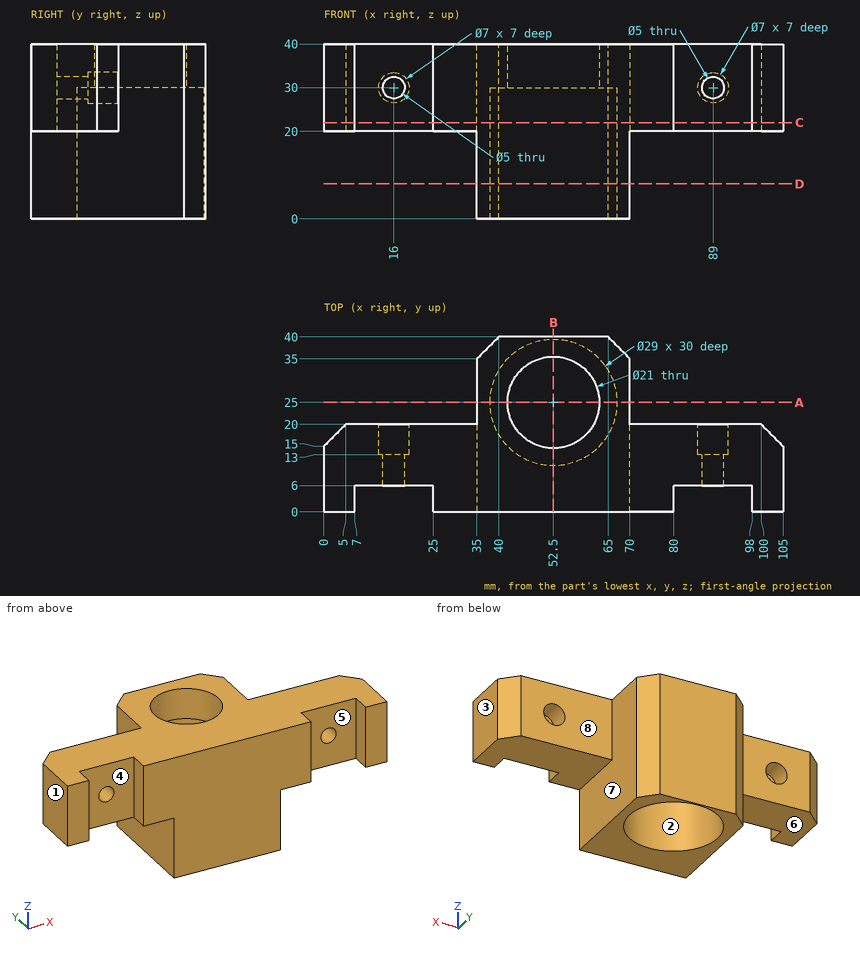
Check sheet for the drawn part. Datum: minimum x, y, z corner. Units: mm. A direction names the side the tool comes from. Round coordinates to 2 decimals unless told otherwise and drop trailing zeros. Order: outer loops, then holes, each group sorted by start corner. A loop starts at its lowest first (then second) coordinate and runs counter-clockwise, first axis right, second up.
1. Access from +Z, -Z, +X, -X, +Y, -Y to the whole of each face (thin tool, end or side, straight path). Record for the marked faces 5, 6, 7 and 8.
Final values:
face 5: +Z, -Z, -Y
face 6: -Z, -X, +Y, -Y
face 7: -Z, +X, +Y
face 8: +Z, -Z, +X, +Y
2. Section check A-A on y = 25. Record the cut outline in (x, z).
Final values:
outline: (35, 0) - (38, 0) - (38, 30) - (42, 30) - (42, 40) - (35, 40) - close; (63, 30) - (67, 30) - (67, 0) - (70, 0) - (70, 40) - (63, 40) - close
3. Section check D-D on z = 8. Record the cut outline in (x, y), then the cut area to 3 significant figures.
Final values:
outline: (35, 0) - (70, 0) - (70, 35) - (65, 40) - (40, 40) - (35, 35) - close; hole circle Ø29 at (52.5, 25)
area: 714 mm2
4. Section check B-B on x = 52.5. Record the cut outline in (y, z), then the cut area to 3 significant figures.
Final values:
outline: (0, 0) - (10.5, 0) - (10.5, 30) - (14.5, 30) - (14.5, 40) - (0, 40) - close; (35.5, 30) - (39.5, 30) - (39.5, 0) - (40, 0) - (40, 40) - (35.5, 40) - close
area: 520 mm2
5. Release check for a two-part mould opening along X. For the marked faces 1, 2, 3 and 4 record: +X half, -X half, draft (parallel to the pull), parting line (faces both ways), or undercut.
Final values:
face 1: -X half
face 2: undercut
face 3: +X half
face 4: undercut
6. Thickness scan on L1, parallel to Y at x = 52, z = 6; L2, parallel to Z at x = 89, y = 10; L3, parallel to Y at x = 52, z = 33. Record the ranges inside material, lowest first.
Final values:
L1: y = 0 to 10.51, 39.49 to 40
L2: z = 20 to 27.5, 32.5 to 40
L3: y = 0 to 14.51, 35.49 to 40
7. Go/stop test with flat-tipped pins: P1, Ø5, axis at x = 11.5, y = 8.5, coming from the -Z side; P2, Ø12, axis at x = 18.5, z = 28.5, coming from the -Y side; P3, Ø9, axis at x = 89, z = 30, coming from the +Y side. Record where each tip stops, or that it passes through.
Final values:
P1: stops at z = 20
P2: stops at y = 6
P3: stops at y = 20
8. Section check C-C on z = 22. Record the cut outline in (x, y), then the cut area to 3 significant figures.
Final values:
outline: (0, 0) - (7, 0) - (7, 6) - (25, 6) - (25, 0) - (80, 0) - (80, 6) - (98, 6) - (98, 0) - (105, 0) - (105, 15) - (100, 20) - (70, 20) - (70, 35) - (65, 40) - (40, 40) - (35, 35) - (35, 20) - (5, 20) - (0, 15) - close; hole circle Ø29 at (52.5, 25)
area: 1,870 mm2
